Source: CAD feature listing. Evaluate the final solid. Frame: model axes, mm. Face numbers are marked on the shaded views. A direction names the side the tool comes from. Round coordinates to 2 decimals unless told otherwise and drop trailing zeros. Loops run counter-clockwise (first coordinate to the right, second up) from the corner with the lowest first, then second, coordinate; pieces in that order, holes last. Notation, with made-up numbers: (-12, 56) -> (-2, 56) arc R8 cw to (-2, 61) -> close; hole circle Ø8 at (-22.5, 76). An arc over 180 degrees is marked (long way). Return JSON: item names as keys, results as strings. Group by question number.
```python
from build123d import *

# Parameters (mm, degrees)
SKETCH_2_W          = 170
SKETCH_2_H          = 110
EXTRUDE_2_DEPTH     = 500
SKETCH_5_OUTSIDE_W  = 609.888
SKETCH_5_OUTSIDE_H  = 219.888
CUT_EXTRUDE_3_DEPTH = 200
FILLET_2_R          = 10
SHELL_2_T           = -12


with BuildPart() as part:
    # 草图2 → 凸台-拉伸2 (new body)
    with BuildSketch(Plane.XY):
        Rectangle(SKETCH_2_W, SKETCH_2_H)
    extrude(amount=EXTRUDE_2_DEPTH)

    # 草图5 outside → 切除-拉伸3 (cut)
    with BuildSketch(Plane.ZY.offset(85)):
        with Locations((250, 0)):
            Rectangle(SKETCH_5_OUTSIDE_W, SKETCH_5_OUTSIDE_H)
        Polygon((386.948309985, 55), (386.948309985, -55), (203.948309985, 55), align=None, mode=Mode.SUBTRACT)
    extrude(amount=-CUT_EXTRUDE_3_DEPTH, mode=Mode.SUBTRACT)

    # 圆角2
    fillet_2_edges = [part.edges().sort_by_distance(p)[0] for p in [
        (85, 0, 295.448309985),
        (-85, 0, 295.448309985),
    ]]
    fillet(fillet_2_edges, radius=FILLET_2_R)

    # 抽壳2
    shell_2_openings = [part.faces().sort_by_distance(p)[0] for p in [
        (0, 55, 295.682357503),
        (0, 0.1406843, 386.948309985),
    ]]
    offset(amount=SHELL_2_T, openings=shell_2_openings, kind=Kind.INTERSECTION)


solid = part.part
```
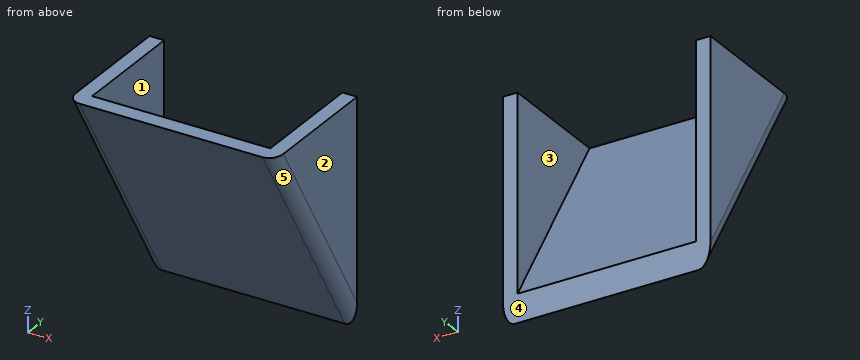
(1) Ray query, line 1 (X direction, y = 15.5, z = 312); line 2 (Z direction, x = 64, y = -21); line 3 (Z direction, x = -48, y = 1). Return the intervals inside material, ascending.
(2) Set-up query: the marked faces 1 and 2. Return all of +Z, -Z, +X, -X, +Y, -Y with unobstructed straight access to the full face (end or side cutting, diameter ignored); none if empty.
(3) Mould query, pull axis X, two halves, no side actions, for the marked faces 3, 4 and 5. Classes: released by +X, released by -X, zero draft, split by the parting line, or undercut.
(4) Pin query (flat end, axial travel): pin 1 (2 mm diameter, centred on y = 5.5, z = 295.5, fed in from -X); pin 2 (10 mm diameter, centred on x = -13, y = -5, fed in from +Z); pin 3 (6 mm diameter, centred on x = 65, z = 362.5, fed in from +Y). Return the tip coordinate at first contact, or that it passes through.
(5) Cut plane A-A (x = -70.5). Return loops of the section in (y, z).
Answers follow:
{
 "1": {"line 1": "-85 to -73, 73 to 85", "line 2": "330.38 to 353.68", "line 3": "293.78 to 317.08"},
 "2": {"face 1": "+Z, +Y", "face 2": "+Z, -Z, +X, +Y, -Y"},
 "3": {"face 3": "undercut", "face 4": "zero draft", "face 5": "released by +X"},
 "4": {"pin 1": "x = -84.05", "pin 2": "z = 335.38", "pin 3": "y = -24.5"},
 "5": {"outline": "(-55, 386.95) -> (55, 203.95) -> (55, 227.24) -> (-41, 386.95) -> close"}
}
